from build123d import *

# Parameters (mm, degrees)
SKETCH2_W           = 150
SKETCH2_H           = 25
BOSS_EXTRUDE1_DEPTH = 15
SKETCH3_R           = 30
BOSS_EXTRUDE2_DEPTH = 30
SKETCH4_R           = 5.5
CUT_EXTRUDE1_DEPTH  = 30
BOSS_EXTRUDE3_START = -30
SKETCH5_R           = 30
BOSS_EXTRUDE3_DEPTH = 150


with BuildPart() as part:
    # Sketch2 → Boss-Extrude1 (new, symmetric)
    with BuildSketch(Plane.XY):
        Rectangle(SKETCH2_W, SKETCH2_H)
    extrude(amount=BOSS_EXTRUDE1_DEPTH, both=True)

    # Sketch3 → Boss-Extrude2 (add)
    with BuildSketch(Plane.XY.offset(15)):
        with BuildLine():
            Line((-15, 87.5), (-15, 0))
            Line((-15, 0), (75, 0))
            Line((75, 0), (75, 87.5))
            ThreePointArc((75, 87.5), (30, 132.5), (-15, 87.5))
        make_face()
        with Locations((30, 87.5)):
            Circle(SKETCH3_R, mode=Mode.SUBTRACT)
    extrude(amount=-BOSS_EXTRUDE2_DEPTH)

    # Sketch4 → Cut-Extrude1 (cut)
    with BuildSketch(Plane(origin=(0, 12.5, 0), x_dir=(1, 0, 0), z_dir=(0, 1, 0))):
        with Locations(Location((-60, 0, 0), (0, 0, 270))):
            Circle(SKETCH4_R)
        with Locations(Location((-40, 0, 0), (0, 0, 270))):
            Circle(SKETCH4_R)
    extrude(amount=-CUT_EXTRUDE1_DEPTH, mode=Mode.SUBTRACT)

    # Sketch5 → Boss-Extrude3 (add)
    with BuildSketch(Plane(origin=(0, 0, -15), x_dir=(-1, 0, 0), z_dir=(0, 0, -1)).offset(BOSS_EXTRUDE3_START)):
        with Locations(Location((-30, 87.5, 0), (0, 0, 180))):
            Circle(SKETCH5_R)
    extrude(amount=BOSS_EXTRUDE3_DEPTH)


solid = part.part
For this review, take the finished solid that the model builds, in its own axes (mm). A direction names the side the tool comes from. Coordinates: 2 decimals unless noted, no trailing zeros. Loops run counter-clockwise (first coordinate to the right, second up) from the corner with the lowest first, then second, coordinate; pieces in that order, holes last. Notation, with made-up numbers: (-16, 27) - (11, 27) arc R18 cw to (11, 32) - close; hole circle Ø11 at (7, -30). An arc over 180 degrees is marked (long way). Use a Markdown table: item, result. Add a question column.
Item 1: Tool access review of faces 1 (the face through (7.889, 67.225, -74.16)), 2 (the face through (30, 87, -135)), 3 (the face through (-45, 12.5, 4)): name each direction out of +Z, -Z, +X, -X, +Y, -Y from which nothing blocks a thin tool from reaching the whole face with its end or side.
Item 2: We need section C-C (y = 1). Give the boundary of the cut face in (x, z).
Item 3: Insertion check: pin 1 Ø12 at (y, z) = (91.5, -32.5) entering from +X; pin 2 Ø9 at (x, z) = (-47.5, -5) entering from +Y; pin 3 Ø9 at (y, z) = (44.5, 5.5) entering from -X. Each pin has a flat end and moves straight along its axis. Give the tip position at first contact, or say it passes through.
Item 4: We need section D-D (x = 30). Give the boundary of the cut face in (y, z).
Item 5: We need section A-A (x = -60). Give the boundary of the cut face in (y, z).
Item 6: We need section B-B (z = 0). Give the boundary of the cut face in (x, y), and give its area (3 significant figures).
Item 7: For line 1 (X direction, y = 5.75, z = 0); line 2 (Y direction, x = 28.5, z = -115.5); line 3 (X direction, y = 15, z = 3), list the stretches that pass through material, from the lowest coordinate up.
Results list:
| question | item | result |
|---|---|---|
| 1 | face 1 | -Z |
| 1 | face 2 | -Z, +X, -X, +Y, -Y |
| 1 | face 3 | +Z, -Z, -X, +Y |
| 2 | outline | (-75, -15) - (75, -15) - (75, 15) - (-75, 15) - close; hole circle Ø11 at (-60, 0); hole circle Ø11 at (-40, 0) |
| 3 | pin 1 | stops at x = 60 |
| 3 | pin 2 | stops at y = 12.5 |
| 3 | pin 3 | stops at x = -15 |
| 4 | outline | (-12.5, -15) - (57.5, -15) - (57.5, -135) - (117.5, -135) - (117.5, -15) - (132.5, -15) - (132.5, 15) - (-12.5, 15) - close |
| 5 | outline | (-12.5, -15) - (12.5, -15) - (12.5, -5.5) - (-12.5, -5.5) - close; (-12.5, 5.5) - (12.5, 5.5) - (12.5, 15) - (-12.5, 15) - close |
| 6 | outline | (-75, -12.5) - (-65.5, -12.5) - (-65.5, 12.5) - (-75, 12.5) - close; (-54.5, -12.5) - (-45.5, -12.5) - (-45.5, 12.5) - (-54.5, 12.5) - close; (-34.5, -12.5) - (75, -12.5) - (75, 87.5) arc R45 ccw to (-15, 87.5) - (-15, 12.5) - (-34.5, 12.5) - close |
| 6 | area | 13,100 mm^2 |
| 7 | line 1 | x = -75 to -65.5, -54.5 to -45.5, -34.5 to 75 |
| 7 | line 2 | y = 57.54 to 117.46 |
| 7 | line 3 | x = -15 to 75 |
